```python
from build123d import *

# Parameters (mm, degrees)
SKETCH1_W           = 120
SKETCH1_H           = 80
BOSS_EXTRUDE1_DEPTH = 1002
FILLET1_R           = 10
SHELL1_T            = -4


with BuildPart() as part:
    # Sketch1 → Boss-Extrude1 (new body)
    with BuildSketch(Plane.XY):
        Rectangle(SKETCH1_W, SKETCH1_H)
    extrude(amount=BOSS_EXTRUDE1_DEPTH)

    # Fillet1
    fillet1_edges = [part.edges().sort_by_distance(p)[0] for p in [
        (-60, 40, 501),
        (60, 40, 501),
        (60, -40, 501),
        (-60, -40, 501),
    ]]
    fillet(fillet1_edges, radius=FILLET1_R)

    # Shell1
    shell1_openings = [part.faces().sort_by_distance(p)[0] for p in [
        (0, 0, 1002),
        (0, 0, 0),
    ]]
    offset(amount=SHELL1_T, openings=shell1_openings, kind=Kind.INTERSECTION)


solid = part.part
```
Source: CAD feature listing. Evaluate the final solid. Frame: model axes, mm. A direction names the side the tool comes from. Round coordinates to 2 decimals unless told otherwise and drop trailing zeros. Loops run counter-clockwise (first coordinate to the right, second up) from the corner with the lowest first, then second, coordinate; pieces in that order, holes last. Notation, with made-up numbers: M -32,-24 L 7,-24 A29 cw 7,-4 Z; hole C 27,41.5 d7. An arc over 180 degrees is marked long. Use a Markdown table: item, result. Add a question column.
1. Mould query, pull axis X, two halves, no side actions, for faces 1 (the flat face through (-1, 40, 494)), 2 (the flat face through (60, 0, 494)), 3 (the flat face through (-1, -36, 494)). Classes: pulls with the +X half, pulls with the -X half, needs draft (parallel to the pull), parting line crosses it, or undercut.
2. Line query: line 1 (Y direction, x = -27, z = 485.5); line 2 (X direction, y = 25.5, z = 48); line 3 (X direction, y = -34, z = 769). Output: solid intervals per line, ascending.
3. Section query B-B on x = 34. Return the cut outline in (y, z), then the cut area to 3 significant figures.
4. Section query A-A on y = -0.5. Return the cut outline in (x, z), then the cut area to 3 significant figures.
5. Section query C-C on z = 801.5. Return the cut outline in (x, y).
6. Reachability of faces 4 (the flat face through (-56, 0, 494)), 5 (the flat face through (-5, -38, 0)) from +Z, -Z, +X, -X, +Y, -Y: full face, straight path, thin tool, end or side. Return the list, or none.
Reported:
| question | item | result |
|---|---|---|
| 1 | face 1 | needs draft |
| 1 | face 2 | pulls with the +X half |
| 1 | face 3 | undercut |
| 2 | line 1 | y = -40 to -36, 36 to 40 |
| 2 | line 2 | x = -60 to -56, 56 to 60 |
| 2 | line 3 | x = -59.17 to -54.47, 54.47 to 59.17 |
| 3 | outline | M -40,0 L -36,0 L -36,1002 L -40,1002 Z; M 36,0 L 40,0 L 40,1002 L 36,1002 Z |
| 3 | area | 8,020 mm² |
| 4 | outline | M -60,0 L -56,0 L -56,1002 L -60,1002 Z; M 56,0 L 60,0 L 60,1002 L 56,1002 Z |
| 4 | area | 8,020 mm² |
| 5 | outline | M -60,-30 A10 ccw -50,-40 L 50,-40 A10 ccw 60,-30 L 60,30 A10 ccw 50,40 L -50,40 A10 ccw -60,30 Z; hole M -56,-30 A6 ccw -50,-36 L 50,-36 A6 ccw 56,-30 L 56,30 A6 ccw 50,36 L -50,36 A6 ccw -56,30 Z |
| 6 | face 4 | +Z, -Z |
| 6 | face 5 | -Z, +X, -X, +Y, -Y |
